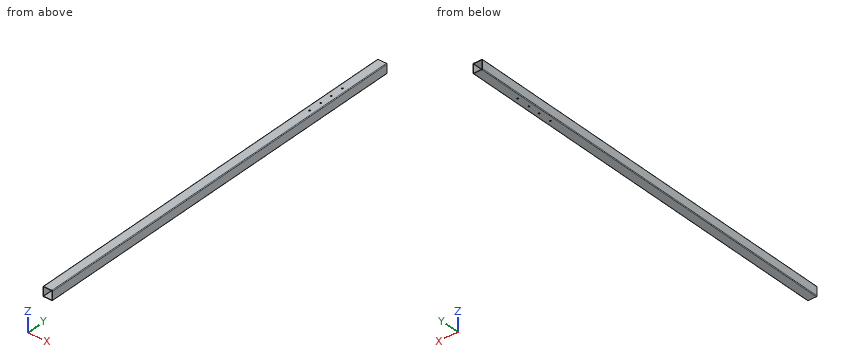
```python
from build123d import *

# Parameters (mm, degrees)
BOSS_EXTRUDE1_DEPTH     = 2097
CUT_EXTRUDE1_DEPTH      = 2098.744979734
CUT_EXTRUDE1_DEPTH_BACK = 2098.744979734
SKETCH2_R               = 4


with BuildPart() as part:
    # Sketch1 → Boss-Extrude1 (new body)
    with BuildSketch(Plane(origin=(0, 0, 0), x_dir=(1, 0, 0), z_dir=(0, 1, 0))):
        with BuildLine():
            Line((-21.55, -25), (21.55, -25))
            ThreePointArc((21.55, -25), (23.989518395, -23.989518395), (25, -21.55))
            Line((25, -21.55), (25, 21.55))
            ThreePointArc((25, 21.55), (23.989518395, 23.989518395), (21.55, 25))
            Line((21.55, 25), (-21.55, 25))
            ThreePointArc((-21.55, 25), (-23.989518395, 23.989518395), (-25, 21.55))
            Line((-25, 21.55), (-25, -21.55))
            ThreePointArc((-25, -21.55), (-23.989518395, -23.989518395), (-21.55, -25))
        make_face()
        with BuildLine():
            Line((-21.55, -22.7), (21.55, -22.7))
            ThreePointArc((21.55, -22.7), (22.363172798, -22.363172798), (22.7, -21.55))
            Line((22.7, -21.55), (22.7, 21.55))
            ThreePointArc((22.7, 21.55), (22.363172798, 22.363172798), (21.55, 22.7))
            Line((21.55, 22.7), (-21.55, 22.7))
            ThreePointArc((-21.55, 22.7), (-22.363172798, 22.363172798), (-22.7, 21.55))
            Line((-22.7, 21.55), (-22.7, -21.55))
            ThreePointArc((-22.7, -21.55), (-22.363172798, -22.363172798), (-21.55, -22.7))
        make_face(mode=Mode.SUBTRACT)
    extrude(amount=BOSS_EXTRUDE1_DEPTH)

    # Sketch2 → Cut-Extrude1 (cut, two sides: drawn at the far end of the back side and taken through both)
    with BuildSketch(Plane(origin=(0, 0, -25), x_dir=(-1, 0, 0), z_dir=(0, 0, -1)).offset(-CUT_EXTRUDE1_DEPTH_BACK)):
        with Locations(Location((0, 1847, 0), (0, 0, 180))):
            Circle(SKETCH2_R)
        with Locations(Location((0, 1777, 0), (0, 0, 180))):
            Circle(SKETCH2_R)
        with Locations(Location((0, 1712, 0), (0, 0, 180))):
            Circle(SKETCH2_R)
        with Locations(Location((0, 1642, 0), (0, 0, 180))):
            Circle(SKETCH2_R)
    extrude(amount=CUT_EXTRUDE1_DEPTH + CUT_EXTRUDE1_DEPTH_BACK, mode=Mode.SUBTRACT)


solid = part.part
```
Geometry check sheet. Reference: the model listing, model coordinates, mm. Round coordinates to 2 decimals unless told otherwise and drop trailing zeros. Write each loop counter-clockwise with the first axis right and the second up, starting at its lowest first coordinate (ties: lowest second). Pieces come first, ordered by that corner, then holes. Notation, with made-up numbers: (73.25, 38.5) - (127.25, 38.5) arc R5 ccw to (127.25, 42.5) - close; hole circle Ø6 at (43, 51). An arc over 180 degrees is marked (long way). Write each question's results on one line, items separated by ' | '.
(1) Sectioned sample at B-B, the plane y = 410.5. Enter the section's corners in (x, z).
Computed:
outline: (-25, -21.55) arc R3.45 ccw to (-21.55, -25) - (21.55, -25) arc R3.45 ccw to (25, -21.55) - (25, 21.55) arc R3.45 ccw to (21.55, 25) - (-21.55, 25) arc R3.45 ccw to (-25, 21.55) - close; hole (-22.7, -21.55) arc R1.15 ccw to (-21.55, -22.7) - (21.55, -22.7) arc R1.15 ccw to (22.7, -21.55) - (22.7, 21.55) arc R1.15 ccw to (21.55, 22.7) - (-21.55, 22.7) arc R1.15 ccw to (-22.7, 21.55) - close
(2) Sectioned sample at A-A, the plane z = 9. Enter the section's corners in (x, y), plus the area to 3 significant figures.
Computed:
outline: (-25, 0) - (-22.7, 0) - (-22.7, 2097) - (-25, 2097) - close; (22.7, 0) - (25, 0) - (25, 2097) - (22.7, 2097) - close | area: 9,650 mm^2
(3) Thickness scan on probe 1 along Y at (x, z) = (0, -23.4); probe 2 along Z at (x, y) = (-6, 184.5). Record the ranges inside material, lowest first. Write a range as from..to.
Computed:
probe 1: y = 0..1638, 1646..1708, 1716..1773, 1781..1843, 1851..2097 | probe 2: z = -25..-22.7, 22.7..25
